Check sheet for the modelled part. Datum: model origin and axes. Units: mm. A direction names the side the tool comes from. Give positions to 0.01 mm unless a question says otherwise; leave off trailing zeros. Order: outer loops, then holes, each group sorted by start corner. A loop starts at its lowest first (then second) coordinate and runs counter-clockwise, first axis right, second up.
Item 1: Release check for a two-part mould opening along X. For faces 4 (the cylindrical face through (14.1, 4, 3.4)), 5 (the flat face through (-6.5, -2.4, -2.4)), 6 (the flat face through (-21.5, -2.3, -2.4)) record: released by +X, released by -X, zero draft, split by the parting line, or undercut.
Item 2: Sectioned sample at C-C on z = 1. Record the boundary of the cut face in (x, y), and give its area (3 significant figures).
Item 3: Sectioned sample at A-A on y = 0. Record the boundary of the cut face in (x, z), and give its area (3 significant figures).
Item 4: Access from +Z, -Z, +X, -X, +Y, -Y to the whole of each face (thin tool, end or side, straight path). Record for faces 1 (the flat face through (0, -3, -5.5)), 2 (the flat face through (32, -3, -5.5)), 3 (the flat face through (-32, -3, -5.5)).
Item 5: Material ranges on line 1 along X through (y, z) = (-3.5, -4.5); line 2 along Y through (x, z) = (-12.5, 0); line 3 along Y through (x, z) = (-38, -30), recorded low to high.
Item 6: Sectioned sample at B-B on x = -8.5. Record the boundary of the cut face in (y, z).
Item 7: Gauge pin test, flat ends, axial feed: P1, Ø1.5, axis at y = 0, z = -2, coming from the -X side; P2, Ø1.2, axis at x = -30, y = -2.5, coming from the +Z side; P3, Ø14, axis at x = -10.5, z = -13.5, coming from the +Y side; P4, Ø5, axis at y = 0.5, z = 1.5, coming from the +X side. Record the tip position at first contact, or that the pin passes through.
Item 8: Sectioned sample at D-D on z = -13. Record the boundary of the cut face in (x, y).
from build123d import *

# Parameters (mm, degrees)
BOSS_EXTRUDE1_DEPTH = 42.5
SKETCH3_W           = 13
SKETCH3_H           = 11
SKETCH3_W_2         = 21
SKETCH3_H_2         = 10.75
CUT_EXTRUDE2_DEPTH  = 10
SKETCH4_R           = 3
CUT_EXTRUDE3_DEPTH  = 73.198078229


with BuildPart() as part:
    # Sketch1 → Boss-Extrude1 (new, symmetric)
    with BuildSketch(Plane(origin=(0, 0, 0), x_dir=(0, 0, -1), z_dir=(1, 0, 0))):
        with BuildLine():
            Line((33, -5.25), (0, -5.25))
            ThreePointArc((0, -5.25), (-3.240370349, 4.13067791), (5.099019514, -1.25))
            Line((5.099019514, -1.25), (33, -1.25))
            Line((33, -1.25), (33, -5.25))
        make_face()
    extrude(amount=BOSS_EXTRUDE1_DEPTH, both=True)

    # Sketch3 → Cut-Extrude2 (cut, symmetric)
    with BuildSketch(Plane(origin=(0, 0, 0), x_dir=(1, 0, 0), z_dir=(0, 1, 0))):
        Rectangle(SKETCH3_W, SKETCH3_H)
        with Locations((32, 0.125)):
            Rectangle(SKETCH3_W_2, SKETCH3_H_2)
        with Locations((-32, 0.125)):
            Rectangle(SKETCH3_W_2, SKETCH3_H_2)
    extrude(amount=CUT_EXTRUDE2_DEPTH, both=True, mode=Mode.SUBTRACT)

    # Sketch4 → Cut-Extrude3 (cut, through all)
    with BuildSketch(Plane.ZY.offset(21.5)):
        Circle(SKETCH4_R)
    extrude(amount=-CUT_EXTRUDE3_DEPTH, mode=Mode.SUBTRACT)


solid = part.part
Report:
1. face 4: zero draft
1. face 5: undercut
1. face 6: released by -X
2. outline: (-21.5, -5.15) - (-6.5, -5.15) - (-6.5, -2.83) - (-21.5, -2.83) - close; (-21.5, 2.83) - (-6.5, 2.83) - (-6.5, 5.15) - (-21.5, 5.15) - close; (6.5, -5.15) - (21.5, -5.15) - (21.5, -2.83) - (6.5, -2.83) - close; (6.5, 2.83) - (21.5, 2.83) - (21.5, 5.15) - (6.5, 5.15) - close
2. area: 140 mm2
3. outline: (-21.5, -5.25) - (-6.5, -5.25) - (-6.5, -3) - (-21.5, -3) - close; (-21.5, 3) - (-6.5, 3) - (-6.5, 5.25) - (-21.5, 5.25) - close; (6.5, -5.25) - (21.5, -5.25) - (21.5, -3) - (6.5, -3) - close; (6.5, 3) - (21.5, 3) - (21.5, 5.25) - (6.5, 5.25) - close
3. area: 135 mm2
4. face 1: +Z, +Y, -Y
4. face 2: +Z, +X, +Y, -Y
4. face 3: +Z, -X, +Y, -Y
5. line 1: x = -21.5 to -6.5, 6.5 to 21.5
5. line 2: y = -5.25 to -3, 3 to 5.25
5. line 3: y = -5.25 to -1.25
6. outline: (-5.25, -33) - (-1.25, -33) - (-1.25, -5.1) arc R5.25 ccw (long way) to (-5.25, 0) - close; hole circle Ø6 at (0, 0)
7. P1: passes through
7. P2: stops at z = -5.5
7. P3: stops at y = -1.25
7. P4: stops at x = 21.5
8. outline: (-42.5, -5.25) - (42.5, -5.25) - (42.5, -1.25) - (-42.5, -1.25) - close
